Can you work these out from the model? Positions are in its coordinate system, mm. A direction names the side the tool comes from. Give positions to 0.01 mm unless a question says otherwise; leave off trailing zeros. Write each loop counter-clockwise with the first axis right and the second up, starting at its lowest first coordinate (ties: lowest second). Pieces come first, ordered by that corner, then holes. Notation, with made-up numbers: (-1, -7.5) - (49, -7.5) arc R19 ccw to (49, 19.5) - close; hole circle Ø10 at (23.25, 72.5). An arc over 180 degrees is marked (long way). Use a Markdown table: item, result. Add a question column.
```python
from build123d import *

# Parameters (mm, degrees)
SKETCH_1_R          = 11
EXTRUDE_1_DEPTH     = 12
SKETCH_2_R          = 2.75
CUT_EXTRUDE_1_DEPTH = 53.135542299
SKETCH_3_R          = 5
CUT_EXTRUDE_2_DEPTH = 5.8


with BuildPart() as part:
    # 草图1 → 凸台-拉伸1 (new body)
    with BuildSketch(Plane.XY):
        Polygon((-16.269702277, -16.03765324), (36.730297723, -16.03765324), (36.730297723, -4.03765324), (24.730297723, -4.03765324), (24.730297723, 30.96234676), (-4.269702277, 30.96234676), (-4.269702277, -4.03765324), (-16.269702277, -4.03765324), align=None)
        with Locations((10.230297723, 13.96234676)):
            Circle(SKETCH_1_R, mode=Mode.SUBTRACT)
    extrude(amount=EXTRUDE_1_DEPTH)

    # 草图2 → 切除-拉伸1 (cut, through all)
    with BuildSketch(Plane(origin=(0, -4.03765324, 0), x_dir=(1, 0, 0), z_dir=(0, 1, 0))):
        with Locations(Location((-10.269702277, -6, 0), (0, 0, 180))):
            Circle(SKETCH_2_R)
        with Locations(Location((30.730297723, -6, 0), (0, 0, 180))):
            Circle(SKETCH_2_R)
    extrude(amount=-CUT_EXTRUDE_1_DEPTH, mode=Mode.SUBTRACT)

    # 草图3 → 切除-拉伸2 (cut)
    with BuildSketch(Plane(origin=(0, -4.03765324, 0), x_dir=(1, 0, 0), z_dir=(0, 1, 0))):
        with Locations(Location((-10.269702277, -6, 0), (0, 0, 180))):
            Circle(SKETCH_3_R)
        with Locations(Location((30.730297723, -6, 0), (0, 0, 180))):
            Circle(SKETCH_3_R)
    extrude(amount=-CUT_EXTRUDE_2_DEPTH, mode=Mode.SUBTRACT)


solid = part.part
```
Q1. Suppose I cut it at B-B (x = 4.5). Please give me the cut outline in (y, z).
Q2. If we mould it in two halves opening along Z, with no side actions, what happens to faces 6 (the flat face through (36, -4.038, 6)), 7 (the cylindrical face through (32.913, -12.894, 4.327)), 8 (the flat face through (9.9, 2.6, 0))? For each: released by +Z, released by -Z, zero draft, split by the parting line, or undercut.
Q3. Suppose I cut it at D-D (y = 27.5). Please give me the cut outline in (x, z).
Q4. If I drill on probe 1 along X at (y, z) = (14.5, 11.25); probe 2 along Y at (x, z) = (26.5, 6); probe 3 along Z at (x, y) = (-11, -13), over which ranges is the centre line in solid material (lowest first)? Write a range as [from, to].
Q5. I'm going to push flat-ended pins straight in: P1, Ø6, axis at y = 17.5, z = 7.5, coming from the -X side; P2, Ø5, axis at x = -10.27, z = 6, coming from the +Y side; P3, Ø5, axis at x = -9, z = 4, coming from the +Y side; P4, Ø6, axis at y = 14, z = 5, coming from the +X side. Where does each tip first touch, or does it pass through?
Q6. Suppose I cut it at A-A (z = 4.75). Please give me the cut outline in (x, y), and give its area (3 significant figures).
Q7. Suppose I cut it at C-C (y = 9). Please give me the cut outline in (x, z).
Q8. On a 3-axis mill with a long thin cutter (end or side, diameter ignored), from which of +Z, -Z, +X, -X, +Y, -Y can I reach the whole of each face in a straight line? I mean faces 1 (the flat face through (24.73, 13, 6)), 2 (the flat face through (9.9, 2.6, 12)), 3 (the flat face through (-4.27, 14, 6)), 4 (the flat face through (-12.4, -9.838, 3.8)), 5 (the flat face through (10, 30.962, 6)). Say none if no direction works.
Derived:
| question | item | result |
|---|---|---|
| 1 | outline | (-16.04, 0) - (4.57, 0) - (4.57, 12) - (-16.04, 12) - close; (23.35, 0) - (30.96, 0) - (30.96, 12) - (23.35, 12) - close |
| 2 | face 6 | zero draft |
| 2 | face 7 | undercut |
| 2 | face 8 | released by -Z |
| 3 | outline | (-4.27, 0) - (24.73, 0) - (24.73, 12) - (-4.27, 12) - close |
| 4 | probe 1 | [-4.27, -0.76], [21.22, 24.73] |
| 4 | probe 2 | [-16.04, -9.84] |
| 4 | probe 3 | [0, 3.35], [8.65, 12] |
| 5 | P1 | x = -4.27 |
| 5 | P2 | through |
| 5 | P3 | y = -9.84 |
| 5 | P4 | x = 24.73 |
| 6 | outline | (-16.27, -16.04) - (-12.72, -16.04) - (-12.72, -9.84) - (-15.11, -9.84) - (-15.11, -4.04) - (-16.27, -4.04) - close; (-7.82, -16.04) - (28.28, -16.04) - (28.28, -9.84) - (25.89, -9.84) - (25.89, -4.04) - (24.73, -4.04) - (24.73, 30.96) - (-4.27, 30.96) - (-4.27, -4.04) - (-5.43, -4.04) - (-5.43, -9.84) - (-7.82, -9.84) - close; (33.18, -16.04) - (36.73, -16.04) - (36.73, -4.04) - (35.57, -4.04) - (35.57, -9.84) - (33.18, -9.84) - close; hole circle Ø22 at (10.23, 13.96) |
| 6 | area | 1,100 mm² |
| 7 | outline | (-4.27, 0) - (0.41, 0) - (0.41, 12) - (-4.27, 12) - close; (20.05, 0) - (24.73, 0) - (24.73, 12) - (20.05, 12) - close |
| 8 | face 1 | +Z, -Z, +X, +Y |
| 8 | face 2 | +Z, +X, -X, +Y, -Y |
| 8 | face 3 | +Z, -Z, -X, +Y |
| 8 | face 4 | +Y |
| 8 | face 5 | +Z, -Z, +X, -X, +Y |
